```python
from build123d import *

# Parameters (mm, degrees)
SKETCH2_W           = 140
SKETCH2_H           = 140
SKETCH2_R           = 9
BOSS_EXTRUDE1_DEPTH = 25


with BuildPart() as part:
    # Sketch1 → Revolve1 (revolve)
    with BuildSketch(Plane.XY, mode=Mode.PRIVATE) as revolve1_sk:
        Polygon((0, 0), (60, 0), (60, 25), (55, 25), (55, 665.5), (51, 665.5), (51, 687), (25, 687), (25, 729), (0, 729), align=None)
    revolve(revolve1_sk.sketch.rotate(Axis((0, 0, 0), (0, -1, 0)), 90), axis=Axis((0, 0, 0), (0, -1, 0)))

    # Sketch2 → Boss-Extrude1 (add)
    with BuildSketch(Plane(origin=(0, 0, 0), x_dir=(1, 0, 0), z_dir=(0, 1, 0))):
        Rectangle(SKETCH2_W, SKETCH2_H)
        with Locations(Location((-55.5, 55.5, 0), (0, 0, 270))):
            Circle(SKETCH2_R, mode=Mode.SUBTRACT)
        with Locations(Location((55.5, 55.5, 0), (0, 0, 270))):
            Circle(SKETCH2_R, mode=Mode.SUBTRACT)
        with Locations(Location((55.5, -55.5, 0), (0, 0, 270))):
            Circle(SKETCH2_R, mode=Mode.SUBTRACT)
        with Locations(Location((-55.5, -55.5, 0), (0, 0, 270))):
            Circle(SKETCH2_R, mode=Mode.SUBTRACT)
    extrude(amount=BOSS_EXTRUDE1_DEPTH)


solid = part.part
```
Could you check a few things on this model? Use its own coordinates, in mm. A direction names the side the tool comes from. Round coordinates to 2 decimals unless told otherwise and drop trailing zeros. Loops run counter-clockwise (first coordinate to the right, second up) from the corner with the lowest first, then second, coordinate; pieces in that order, holes last. Notation, with made-up numbers: (-20, 39.25) -> (19, 39.25) arc R8 cw to (19, 43.25) -> close; hole circle Ø5 at (18, 64). An arc over 180 degrees is marked (long way). Put each result on its own line as item: value.
Q1. For pin 1 Ø10 at (y, z) = (339.5, -56) entering from +X; pin 2 Ø8 at (x, z) = (26, 17.5) entering from +Y; pin 3 Ø23.5 at (x, z) = (55.5, -55.5) entering from +Y; pin 4 Ø4 at (x, z) = (-51, 22.5) entering from -Y, each with a flat end and sliding along its axis, tell me the tip position at first contact or that it passes through.
Checks:
pin 1: x = 20.59
pin 2: y = 687
pin 3: y = 25
pin 4: y = 0
Q2. I want a section at D-D on z = -39. Write out the boundary of the cut face in (x, y).
Checks:
outline: (-70, 0) -> (70, 0) -> (70, 25) -> (38.78, 25) -> (38.78, 665.5) -> (32.86, 665.5) -> (32.86, 687) -> (-32.86, 687) -> (-32.86, 665.5) -> (-38.78, 665.5) -> (-38.78, 25) -> (-70, 25) -> close
Q3. Please list where these lines run through material, in increasing order: line 1 (X direction, y = 16, z = 55); line 2 (X direction, y = 71, z = 2.5). Write a range as from..to.
Checks:
line 1: -70..-64.49, -46.51..46.51, 64.49..70
line 2: -54.94..54.94
Q4. I want a section at A-A on x = 0. Write out the boundary of the cut face in (y, z), and give its area (3 significant figures).
Checks:
outline: (0, -70) -> (25, -70) -> (25, -55) -> (665.5, -55) -> (665.5, -51) -> (687, -51) -> (687, -25) -> (729, -25) -> (729, 25) -> (687, 25) -> (687, 51) -> (665.5, 51) -> (665.5, 55) -> (25, 55) -> (25, 70) -> (0, 70) -> close
area: 78,200 mm2
Q5. I want a section at C-C on y = 432.5. Write out the boundary of the cut face in (x, z), and give its area (3 significant figures).
Checks:
outline: circle Ø110 at (0, 0)
area: 9,500 mm2
Q6. Which directions (+Z, -Z, +X, -X, +Y, -Y) give clear straight access to the entire face, cutting with the end or side of a thin tool? Please do faces 4 (the flat face through (-1, 0, -1)), 5 (the cylindrical face through (48.794, 349.734, 25.379)).
Checks:
face 4: +Z, -Z, +X, -X, -Y
face 5: +Y
Q7. Thinking about a two-plate mould opening in Z: for faces 1 (the flat face through (49, 665.5, 16)), 2 (the cylindrical face through (-52.797, 12.325, -46.916)), 3 (the cylindrical face through (-7.509, 708.294, 23.846)), which applies, pulls with the +Z half, pulls with the -Z half, needs draft (parallel to the pull), parting line crosses it, or undercut?
Checks:
face 1: needs draft
face 2: undercut
face 3: parting line crosses it
Q8. I want a section at B-B on z = 0. Write out the boundary of the cut face in (x, y), and give its area (3 significant figures).
Checks:
outline: (-70, 0) -> (70, 0) -> (70, 25) -> (55, 25) -> (55, 665.5) -> (51, 665.5) -> (51, 687) -> (25, 687) -> (25, 729) -> (-25, 729) -> (-25, 687) -> (-51, 687) -> (-51, 665.5) -> (-55, 665.5) -> (-55, 25) -> (-70, 25) -> close
area: 78,200 mm2
